Design review of the part built by this model. Coordinates are the model's own, in mm. Round coordinates to 2 decimals unless told otherwise and drop trailing zeros. Order: outer loops, then holes, each group sorted by start corner. A loop starts at its lowest first (then second) coordinate and runs counter-clockwise, first axis right, second up.
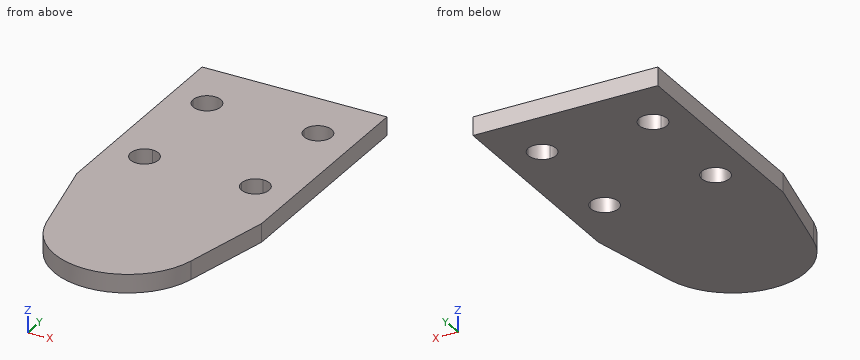
from build123d import *

# Parameters (mm, degrees)
SKETCH_1_R          = 20
EXTRUDE_1_DEPTH     = 10
CUT_EXTRUDE_1_DEPTH = 10
EXTRUDE_START       = -10
EXTRUDE_4_DEPTH     = 10
EXTRUDE_8_DEPTH     = 10
SKETCH_5_R          = 22.505017269
EXTRUDE_9_DEPTH     = 10


with BuildPart() as part:
    # Sketch 1 → Extrude 1 (new body)
    with BuildSketch(Plane.XY):
        with BuildLine():
            Line((0, 0), (90, 0))
            Line((90, 0), (84.980633901, -161.244553285))
            ThreePointArc((84.980633901, -161.244553285), (45, -200), (5.019366099, -161.244553285))
            Line((5.019366099, -161.244553285), (0, 0))
        make_face()
        with Locations((45, -160)):
            Circle(SKETCH_1_R, mode=Mode.SUBTRACT)
    extrude(amount=EXTRUDE_1_DEPTH)

    # Sketch 2 → Cut-Extrude 1 (cut)
    with BuildSketch(Plane.XY.offset(10)):
        with BuildLine():
            Line((7.033066451, -30), (14.533066451, -30))
            Line((14.533066451, -30), (22.033066451, -30))
            ThreePointArc((22.033066451, -30), (14.533066451, -22.5), (7.033066451, -30))
        make_face()
        with BuildLine():
            Line((22.033066451, -30), (14.533066451, -30))
            Line((14.533066451, -30), (14.533066451, -37.5))
            ThreePointArc((14.533066451, -37.5), (19.83636731, -35.303300859), (22.033066451, -30))
        make_face()
        with BuildLine():
            Line((14.533066451, -37.5), (14.533066451, -30))
            Line((14.533066451, -30), (7.033066451, -30))
            ThreePointArc((7.033066451, -30), (9.229765592, -35.303300859), (14.533066451, -37.5))
        make_face()
        with BuildLine():
            Line((67.033066451, -30), (74.533066451, -30))
            Line((74.533066451, -30), (82.033066451, -30))
            ThreePointArc((82.033066451, -30), (74.533066451, -22.5), (67.033066451, -30))
        make_face()
        with BuildLine():
            ThreePointArc((67.033066451, -30), (69.229765592, -35.303300859), (74.533066451, -37.5))
            Line((74.533066451, -37.5), (74.533066451, -30))
            Line((74.533066451, -30), (67.033066451, -30))
        make_face()
        with BuildLine():
            Line((74.533066451, -30), (74.533066451, -37.5))
            ThreePointArc((74.533066451, -37.5), (79.83636731, -35.303300859), (82.033066451, -30))
            Line((82.033066451, -30), (74.533066451, -30))
        make_face()
        with BuildLine():
            ThreePointArc((74.533066451, -82.5), (69.229765592, -84.696699141), (67.033066451, -90))
            Line((67.033066451, -90), (74.533066451, -90))
            Line((74.533066451, -90), (74.533066451, -82.5))
        make_face()
        with BuildLine():
            Line((74.533066451, -90), (67.033066451, -90))
            ThreePointArc((67.033066451, -90), (74.533066451, -97.5), (82.033066451, -90))
            ThreePointArc((82.033066451, -90), (79.83636731, -84.696699141), (74.533066451, -82.5))
            Line((74.533066451, -82.5), (74.533066451, -90))
        make_face()
        with BuildLine():
            ThreePointArc((22.033066451, -90), (19.83636731, -84.696699141), (14.533066451, -82.5))
            Line((14.533066451, -82.5), (14.533066451, -90))
            Line((14.533066451, -90), (22.033066451, -90))
        make_face()
        with BuildLine():
            Line((14.533066451, -90), (14.533066451, -82.5))
            ThreePointArc((14.533066451, -82.5), (9.229765592, -95.303300859), (22.033066451, -90))
            Line((22.033066451, -90), (14.533066451, -90))
        make_face()
    extrude(amount=-CUT_EXTRUDE_1_DEPTH, mode=Mode.SUBTRACT)

    # Sketch 3 → Extrude 4 (add)
    with BuildSketch(Plane.XY.offset(10).offset(EXTRUDE_START)):
        with BuildLine():
            Line((5.019366099, -161.244553285), (0, 0))
            Line((0, 0), (0, -120))
            Line((0, -120), (5.275862069, -164.689655172))
            ThreePointArc((5.275862069, -164.689655172), (5.110404302, -162.969874585), (5.019366099, -161.244553285))
        make_face()
        with BuildLine():
            Line((90, 0), (84.980633901, -161.244553285))
            ThreePointArc((84.980633901, -161.244553285), (84.889595698, -162.969874585), (84.724137931, -164.689655172))
            Line((84.724137931, -164.689655172), (90, -120))
            Line((90, -120), (90, 0))
        make_face()
    extrude(amount=EXTRUDE_4_DEPTH)

    # Sketch 4 → Extrude 8 (add)
    with BuildSketch(Plane(origin=(0, 0, 0), x_dir=(-1, 0, 0), z_dir=(0, 0, -1))):
        with BuildLine():
            Line((-90, -120), (-90, 0))
            Line((-90, 0), (-95, 0))
            Line((-95, 0), (-95, -120.294117647))
            Line((-95, -120.294117647), (-84.012960099, -168.831134939))
            ThreePointArc((-84.012960099, -168.831134939), (-84.422970654, -166.769740378), (-84.724137931, -164.689655172))
            Line((-84.724137931, -164.689655172), (-90, -120))
        make_face()
        with BuildLine():
            Line((5, 0), (0, 0))
            Line((0, 0), (0, -120))
            Line((0, -120), (-5.275862069, -164.689655172))
            ThreePointArc((-5.275862069, -164.689655172), (-5.577029346, -166.769740378), (-5.987039901, -168.831134939))
            Line((-5.987039901, -168.831134939), (5, -120.294117647))
            Line((5, -120.294117647), (5, 0))
        make_face()
    extrude(amount=-EXTRUDE_8_DEPTH)

    # Sketch 5 → Extrude 9 (add)
    with BuildSketch(Plane(origin=(0, 0, 0), x_dir=(-1, 0, 0), z_dir=(0, 0, -1))):
        with Locations((-45, -160)):
            Circle(SKETCH_5_R)
    extrude(amount=-EXTRUDE_9_DEPTH)


solid = part.part
1) Clearance check with flat-ended pins moving along their axes: P1, Ø13.5, axis at x = 14.53, y = -90, coming from the +Z side; P2, Ø1.5, axis at y = -137, z = 4.5, coming from the +X side. State where each tip first meets the part, or that it passes through.
Results:
P1: passes through
P2: stops at x = 91.39
2) Take a section at D-D on y = -153.5. Give the boundary of the cut face in (x, z), plus the area to 3 significant figures.
Results:
outline: (2.52, 0) - (87.48, 0) - (87.48, 10) - (2.52, 10) - close
area: 850 mm2
3) Take a section at B-B on x = 72. Give the boundary of the cut face in (y, z), plus the area to 3 significant figures.
Results:
outline: (-189.51, 0) - (-97.06, 0) - (-97.06, 10) - (-189.51, 10) - close; (-82.94, 0) - (-37.06, 0) - (-37.06, 10) - (-82.94, 10) - close; (-22.94, 0) - (0, 0) - (0, 10) - (-22.94, 10) - close
area: 1,610 mm2
4) Take a section at C-C on y = -177. Give the boundary of the cut face in (x, z).
Results:
outline: (8.79, 0) - (81.21, 0) - (81.21, 10) - (8.79, 10) - close
5) To check wall thickness, follow line 1 along X through (y, z) = (-90, 3); line 2 along X through (y, z) = (-85.5, 4.5); line 3 along Y through (x, z) = (74.5, 5.25). State the ranges of each line that lie inside material, in increasing order.
Results:
line 1: x = -5 to 7.03, 22.03 to 67.03, 82.03 to 95
line 2: x = -5 to 8.53, 20.53 to 68.53, 80.53 to 95
line 3: y = -187.01 to -97.5, -82.5 to -37.5, -22.5 to 0
6) Take a section at A-A on z = 5.5. Give the boundary of the cut face in (x, y), plus the area to 3 significant figures.
Results:
outline: (-5, -120.29) - (5.99, -168.83) arc R40 ccw to (84.01, -168.83) - (95, -120.29) - (95, 0) - (-5, 0) - close; hole circle Ø15 at (14.53, -90); hole circle Ø15 at (14.53, -30); hole circle Ø15 at (74.53, -90); hole circle Ø15 at (74.53, -30)
area: 17,500 mm2
